The listing builds one solid part. Answer for the finished solid, in the listing's coordinates (mm). A direction names the side the tool comes from. Coordinates: 2 decimals unless noted, no trailing zeros. Order: outer loops, then holes, each group sorted by start corner. A loop starts at its lowest first (then second) coordinate and runs counter-clockwise, first axis right, second up. Notation, with made-up numbers: (-9.75, 8.25) -> (-2.75, 8.25) arc R17 ccw to (-2.75, 18.25) -> close; hole circle Ø8 at (-37, 64.25). An arc over 180 degrees is marked (long way). Answer in a Markdown table with one row per item.
```python
from build123d import *

# Parameters (mm, degrees)
EXTRUDE_THIN1_DEPTH = 223


with BuildPart() as part:
    # Sketch1 → Extrude-Thin1 (new, symmetric)
    with BuildSketch(Plane(origin=(0, 0, 0), x_dir=(1, 0, 0), z_dir=(0, 1, 0))):
        with BuildLine():
            Line((-40, 25), (40, 25))
            ThreePointArc((40, 25), (47.071067812, 22.071067812), (50, 15))
            Line((50, 15), (50, -15))
            ThreePointArc((50, -15), (47.071067812, -22.071067812), (40, -25))
            Line((40, -25), (-40, -25))
            ThreePointArc((-40, -25), (-47.071067812, -22.071067812), (-50, -15))
            Line((-50, -15), (-50, 15))
            ThreePointArc((-50, 15), (-47.071067812, 22.071067812), (-40, 25))
        make_face()
        with BuildLine():
            Line((-40, 21), (40, 21))
            ThreePointArc((40, 21), (44.242640687, 19.242640687), (46, 15))
            Line((46, 15), (46, -15))
            ThreePointArc((46, -15), (44.242640687, -19.242640687), (40, -21))
            Line((40, -21), (-40, -21))
            ThreePointArc((-40, -21), (-44.242640687, -19.242640687), (-46, -15))
            Line((-46, -15), (-46, 15))
            ThreePointArc((-46, 15), (-44.242640687, 19.242640687), (-40, 21))
        make_face(mode=Mode.SUBTRACT)
    extrude(amount=EXTRUDE_THIN1_DEPTH, both=True)


solid = part.part
```
(1) A cutting plane is placed at A-A, the plane y = 61. Determine the outline of the cut face in (x, z).
Check values:
| item | result |
|---|---|
| outline | (-50, -15) arc R10 ccw to (-40, -25) -> (40, -25) arc R10 ccw to (50, -15) -> (50, 15) arc R10 ccw to (40, 25) -> (-40, 25) arc R10 ccw to (-50, 15) -> close; hole (-46, -15) arc R6 ccw to (-40, -21) -> (40, -21) arc R6 ccw to (46, -15) -> (46, 15) arc R6 ccw to (40, 21) -> (-40, 21) arc R6 ccw to (-46, 15) -> close |
(2) A cutting plane is placed at B-B, the plane x = 26. Determine the outline of the cut face in (y, z), then the cut area to 3 significant figures.
Check values:
| item | result |
|---|---|
| outline | (-223, -25) -> (223, -25) -> (223, -21) -> (-223, -21) -> close; (-223, 21) -> (223, 21) -> (223, 25) -> (-223, 25) -> close |
| area | 3,570 mm² |
(3) Which of the six approach directions +Z, -Z, +X, -X, +Y, -Y give full straight-line access (tool end or side, diameter ignored) to faces 1 (the flat face through (1, 3, 21)), 2 (the flat face through (1, 3, 25))?
Check values:
| item | result |
|---|---|
| face 1 | +Y, -Y |
| face 2 | +Z, +X, -X, +Y, -Y |
(4) For a pull along Z with two mould halves and no side action, classify faces 3 (the flat face through (46, 3, 0)), 4 (the flat face through (-50, 3, 0)), 5 (the cylindrical face through (46.99, 3.12, -22.15)) as released by +Z, released by -Z, zero draft, split by the parting line, or undercut.
Check values:
| item | result |
|---|---|
| face 3 | undercut |
| face 4 | zero draft |
| face 5 | released by -Z |
(5) Find the intervals of material crossed by line 1 along Z through (x, y) = (18.5, -193.5); line 2 along X through (y, z) = (-101, -4.5); line 3 along Z through (x, y) = (-45.5, 23), in increasing order. Write a range as from..to.
Check values:
| item | result |
|---|---|
| line 1 | -25..-21, 21..25 |
| line 2 | -50..-46, 46..50 |
| line 3 | -23.35..-17.4, 17.4..23.35 |
(6) A cutting plane is placed at C-C, the plane z = -10. Determine the outline of the cut face in (x, y).
Check values:
| item | result |
|---|---|
| outline | (-50, -223) -> (-46, -223) -> (-46, 223) -> (-50, 223) -> close; (46, -223) -> (50, -223) -> (50, 223) -> (46, 223) -> close |
